```python
from build123d import *

# Parameters (mm, degrees)
BOSS_EXTRUDE1_DEPTH = 1400


with BuildPart() as part:
    # Sketch1 → Boss-Extrude1 (new body)
    with BuildSketch(Plane.XY):
        with BuildLine():
            Line((6, 0), (44, 0))
            ThreePointArc((44, 0), (48.242640687, 1.757359313), (50, 6))
            Line((50, 6), (50, 44))
            ThreePointArc((50, 44), (48.242640687, 48.242640687), (44, 50))
            Line((44, 50), (6, 50))
            ThreePointArc((6, 50), (1.757359313, 48.242640687), (0, 44))
            Line((0, 44), (0, 6))
            ThreePointArc((0, 6), (1.757359313, 1.757359313), (6, 0))
        make_face()
        with BuildLine():
            Line((6, 45), (44, 45))
            ThreePointArc((44, 45), (44.707106781, 44.707106781), (45, 44))
            Line((45, 44), (45, 6))
            ThreePointArc((45, 6), (44.707106781, 5.292893219), (44, 5))
            Line((44, 5), (6, 5))
            ThreePointArc((6, 5), (5.292893219, 5.292893219), (5, 6))
            Line((5, 6), (5, 44))
            ThreePointArc((5, 44), (5.292893219, 44.707106781), (6, 45))
        make_face(mode=Mode.SUBTRACT)
    extrude(amount=BOSS_EXTRUDE1_DEPTH)


solid = part.part
```
Geometry: final body of the model. Coordinates: model frame, mm. A direction names the side the tool comes from. Round coordinates to 2 decimals unless told otherwise and drop trailing zeros. Order: outer loops, then holes, each group sorted by start corner. A loop starts at its lowest first (then second) coordinate and runs counter-clockwise, first axis right, second up. Notation, with made-up numbers: (-26.5, -13.75) -> (31.5, -13.75) arc R20 cw to (31.5, -3.75) -> close; hole circle Ø5 at (-3, 74.25). An arc over 180 degrees is marked (long way). Use CSV: the item, a comma, the result in double quotes. Start each with the question number.
1) Set-up query: faces 1 (the face through (25, 0, 690)), 2 (the face through (25, 5, 690)). Return all of +Z, -Z, +X, -X, +Y, -Y with unobstructed straight access to the full face (end or side cutting, diameter ignored); none if empty.
2) Draft query along X for faces 3 (the face through (47, 25, 0)), 4 (the face through (0, 25, 690)), 5 (the face through (50, 25, 690)), 6 (the face through (5, 25, 690)). Return one class per face: +X half, -X half, draft (parallel to the pull), parting line (faces both ways), or undercut.
3) Section C-C (z = 1223.5). Return the cut outline in (x, y).
4) First-contact query: pin 1 Ø12 at (x, y) = (16.5, 18.5) entering from +Z; pin 2 Ø10 at (x, y) = (40.5, 34.5) entering from +Z. Flat tips, straight axial feed; report the tip coordinate or a pass-through.
5) Material intervals for line 1 along Y through (x, z) = (22, 1225.5); line 2 along X through (y, z) = (46, 277.5), sorted ascending. Write a range as from..to.
6) Section A-A (x = 35). Return the cut outline in (y, z), and give its area (3 significant figures).
Returned:
1,face 1,"+Z, -Z, +X, -X, -Y"
1,face 2,"+Z, -Z"
2,face 3,"draft"
2,face 4,"-X half"
2,face 5,"+X half"
2,face 6,"undercut"
3,outline,"(0, 6) arc R6 ccw to (6, 0) -> (44, 0) arc R6 ccw to (50, 6) -> (50, 44) arc R6 ccw to (44, 50) -> (6, 50) arc R6 ccw to (0, 44) -> close; hole (5, 6) arc R1 ccw to (6, 5) -> (44, 5) arc R1 ccw to (45, 6) -> (45, 44) arc R1 ccw to (44, 45) -> (6, 45) arc R1 ccw to (5, 44) -> close"
4,pin 1,"passes through"
4,pin 2,"stops at z = 1400"
5,line 1,"y = 0..5, 45..50"
5,line 2,"x = 0.34..49.66"
6,outline,"(0, 0) -> (5, 0) -> (5, 1400) -> (0, 1400) -> close; (45, 0) -> (50, 0) -> (50, 1400) -> (45, 1400) -> close"
6,area,"14,000 mm²"
